from build123d import *

# Parameters (mm, degrees)
SKETCH1_W           = 30
SKETCH1_H           = 40
BOSS_EXTRUDE1_DEPTH = 30
SKETCH2_W           = 27
SKETCH2_H           = 37
CUT_EXTRUDE1_DEPTH  = 62.755555196


with BuildPart() as part:
    # Sketch1 → Boss-Extrude1 (new body)
    with BuildSketch(Plane.XY):
        with Locations((-22.059069992, 19.247597747)):
            Rectangle(SKETCH1_W, SKETCH1_H)
    extrude(amount=BOSS_EXTRUDE1_DEPTH)

    # Sketch2 → Cut-Extrude1 (cut, through all)
    with BuildSketch(Plane.XY.offset(30)):
        with Locations((-22.059069992, 19.247597747)):
            Rectangle(SKETCH2_W, SKETCH2_H)
    extrude(amount=-CUT_EXTRUDE1_DEPTH, mode=Mode.SUBTRACT)


solid = part.part
Source: CAD feature listing. Evaluate the final solid. Frame: model axes, mm. A direction names the side the tool comes from. Give positions to 0.01 mm unless a question says otherwise; leave off trailing zeros. Order: outer loops, then holes, each group sorted by start corner. A loop starts at its lowest first (then second) coordinate and runs counter-clockwise, first axis right, second up. Notation, with made-up numbers: (22, 83) -> (42, 83) arc R25 ccw to (42, 104) -> close; hole circle Ø1 at (70.25, 15.25). An arc over 180 degrees is marked (long way). Write item = value, one per line.
Item 1: Section query C-C (y = 24). Output: boundary loops of the cut face in (x, z).
Check result:
outline = (-37.06, 0) -> (-35.56, 0) -> (-35.56, 30) -> (-37.06, 30) -> close; (-8.56, 0) -> (-7.06, 0) -> (-7.06, 30) -> (-8.56, 30) -> close
Item 2: Section query B-B (z = 14). Output: boundary loops of the cut face in (x, y), then the cut area to 3 significant figures.
Check result:
outline = (-37.06, -0.75) -> (-7.06, -0.75) -> (-7.06, 39.25) -> (-37.06, 39.25) -> close; hole (-35.56, 0.75) -> (-8.56, 0.75) -> (-8.56, 37.75) -> (-35.56, 37.75) -> close
area = 201 mm²
Item 3: Section query A-A (x = -23). Output: boundary loops of the cut face in (y, z), then the cut area to 3 significant figures.
Check result:
outline = (-0.75, 0) -> (0.75, 0) -> (0.75, 30) -> (-0.75, 30) -> close; (37.75, 0) -> (39.25, 0) -> (39.25, 30) -> (37.75, 30) -> close
area = 90.0 mm²
Item 4: Ray query, probe 1 along X at (y, z) = (32, 12); probe 2 along Y at (x, z) = (-23.5, 12.5). Return the intervals inside material, ascending.
Check result:
probe_1 = -37.06 to -35.56, -8.56 to -7.06
probe_2 = -0.75 to 0.75, 37.75 to 39.25
Item 5: Set-up query: faces 1 (the face through (-22, 37.748, 15)), 2 (the face through (-7.059, 19, 15)). Return all of +Z, -Z, +X, -X, +Y, -Y with unobstructed straight access to the full face (end or side cutting, diameter ignored); none if empty.
Check result:
face_1 = +Z, -Z
face_2 = +Z, -Z, +X, +Y, -Y
Item 6: Mould query, pull axis Y, two halves, no side actions, for faces 3 (the face through (-35.559, 19, 15)), 4 (the face through (-22, -0.752, 15)), 5 (the face through (-36.6, 19.3, 0)). Classes: +Y half, -Y half, draft (parallel to the pull), parting line (faces both ways), or undercut.
Check result:
face_3 = undercut
face_4 = -Y half
face_5 = draft
